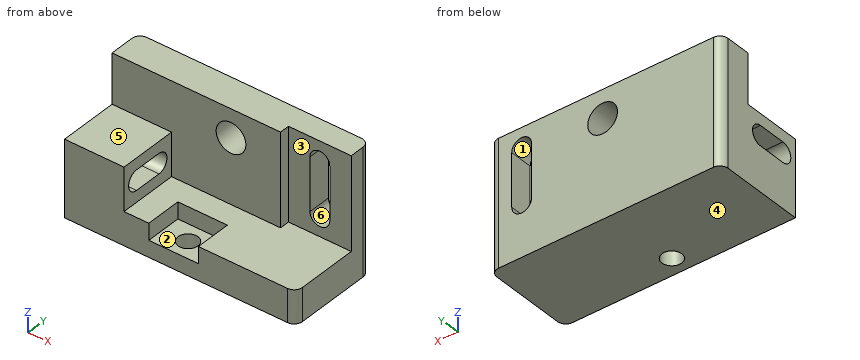
```python
from build123d import *

# Parameters (mm, degrees)
BASE_PLATE_DEPTH             = 76
SIDE_WALL_DEPTH              = 140
POCKET_PROFILE_W             = 38
POCKET_PROFILE_H             = 6
POCKET_CUT_DEPTH             = 56
SLOT_12X32_DEPTH             = 56
GUIDE_START                  = -36
GUIDE_RIB_DEPTH              = 36
OUTER_START                  = -140
OUTER_CORNER_ROUND_R10_DEPTH = 140
RIB_CORNER_ROUND_R10_DEPTH   = 104
CORNER_RELIEF_R10_DEPTH      = 104
HOLE_18_SKETCH_R             = 9
HOLE_18_DEPTH                = 104
NOTCH_PROFILE_W              = 30
NOTCH_PROFILE_H              = 22
NOTCH_CUT_DEPTH              = 10
HOLE_12_SKETCH_R             = 6
HOLE_12_DEPTH                = 10
RIB_SLOT_12_WIDE_DEPTH       = 36


with BuildPart() as part:
    # Base Plate Profile → Base Plate (new body)
    with BuildSketch(Plane.XY):
        with BuildLine():
            Line((5, 0), (135, 0))
            ThreePointArc((135, 0), (138.535533906, -1.464466094), (140, -5))
            Line((140, -5), (140, -20))
            Line((140, -20), (0, -20))
            Line((0, -20), (0, -5))
            ThreePointArc((0, -5), (1.464466094, -1.464466094), (5, 0))
        make_face()
    extrude(amount=BASE_PLATE_DEPTH)

    # Side Wall Profile → Side Wall (add)
    with BuildSketch(Plane(origin=(140, 0, 0), x_dir=(0, 0, -1), z_dir=(1, 0, 0))):
        with BuildLine():
            Line((0, -20), (0, -51))
            ThreePointArc((0, -51), (-1.464466094, -54.535533906), (-5, -56))
            Line((-5, -56), (-15, -56))
            ThreePointArc((-15, -56), (-18.535533906, -54.535533906), (-20, -51))
            Line((-20, -51), (-20, -20))
            Line((-20, -20), (0, -20))
        make_face()
    extrude(amount=-SIDE_WALL_DEPTH)

    # Pocket Profile → Pocket Cut (cut)
    with BuildSketch(Plane.XY.offset(76)):
        with Locations((121, -17)):
            Rectangle(POCKET_PROFILE_W, POCKET_PROFILE_H)
    extrude(amount=-POCKET_CUT_DEPTH, mode=Mode.SUBTRACT)

    # Slot 12x32 Profile → Slot 12x32 (cut)
    with BuildSketch(Plane.XZ.offset(14)):
        with BuildLine():
            Line((115, 64), (115, 32))
            ThreePointArc((115, 32), (121, 26), (127, 32))
            Line((127, 32), (127, 64))
            ThreePointArc((127, 64), (121, 70), (115, 64))
        make_face()
    extrude(amount=-SLOT_12X32_DEPTH, mode=Mode.SUBTRACT)

    # Guide Rib Profile → Guide Rib (add)
    with BuildSketch(Plane.ZY.offset(GUIDE_START)):
        with BuildLine():
            Line((20, -20), (46, -20))
            Line((46, -20), (46, -56))
            Line((46, -56), (15, -56))
            ThreePointArc((15, -56), (18.535533906, -54.535533906), (20, -51))
            Line((20, -51), (20, -20))
        make_face()
    extrude(amount=GUIDE_RIB_DEPTH)

    # Outer Corner Round Profile → Outer Corner Round R10 (add)
    with BuildSketch(Plane.ZY.offset(OUTER_START)):
        with BuildLine():
            Line((0, -51), (0, -56))
            Line((0, -56), (5, -56))
            ThreePointArc((5, -56), (1.464466094, -54.535533906), (0, -51))
        make_face()
    extrude(amount=OUTER_CORNER_ROUND_R10_DEPTH)

    # Rib Corner Round Profile → Rib Corner Round R10 (add)
    with BuildSketch(Plane(origin=(140, 0, 0), x_dir=(0, 0, -1), z_dir=(1, 0, 0))):
        with BuildLine():
            Line((-20, -51), (-20, -56))
            Line((-20, -56), (-15, -56))
            ThreePointArc((-15, -56), (-18.535533906, -54.535533906), (-20, -51))
        make_face()
    extrude(amount=-RIB_CORNER_ROUND_R10_DEPTH)

    # Corner Relief Profile → Corner Relief R10 (cut)
    with BuildSketch(Plane.XY.offset(20)):
        with BuildLine():
            Line((140, -56), (140, -51))
            ThreePointArc((140, -51), (138.535533906, -54.535533906), (135, -56))
            Line((135, -56), (140, -56))
        make_face()
    extrude(amount=-CORNER_RELIEF_R10_DEPTH, mode=Mode.SUBTRACT)

    # Hole Ø18 Sketch → Hole Ø18 (cut)
    with BuildSketch(Plane.XZ.offset(20)):
        with Locations(Location((72, 59, 0), (0, 0, 270))):
            Circle(HOLE_18_SKETCH_R)
    extrude(amount=-HOLE_18_DEPTH, mode=Mode.SUBTRACT)

    # Notch Profile → Notch Cut (cut)
    with BuildSketch(Plane.XY.offset(20)):
        with Locations((66, -45)):
            Rectangle(NOTCH_PROFILE_W, NOTCH_PROFILE_H)
    extrude(amount=-NOTCH_CUT_DEPTH, mode=Mode.SUBTRACT)

    # Hole Ø12 Sketch → Hole Ø12 (cut)
    with BuildSketch(Plane.XY.offset(10)):
        with Locations((66, -45)):
            Circle(HOLE_12_SKETCH_R)
    extrude(amount=-HOLE_12_DEPTH, mode=Mode.SUBTRACT)

    # Rib Slot Profile → Rib Slot 12 Wide (cut)
    with BuildSketch(Plane(origin=(36, 0, 0), x_dir=(0, 0, -1), z_dir=(1, 0, 0))):
        with BuildLine():
            Line((-39, -29.5), (-39, -46.5))
            ThreePointArc((-39, -46.5), (-33, -52.5), (-27, -46.5))
            Line((-27, -46.5), (-27, -29.5))
            ThreePointArc((-27, -29.5), (-33, -23.5), (-39, -29.5))
        make_face()
    extrude(amount=-RIB_SLOT_12_WIDE_DEPTH, mode=Mode.SUBTRACT)


solid = part.part
```
Can you work these out from the model? Positions are in its coordinate system, mm. Face numbers are marked on the shaded views. A direction names the side the tool comes from. Give positions to 0.01 mm unless a question says otherwise; leave off trailing zeros. Write each loop counter-clockwise with the first axis right and the second up, starting at its lowest first coordinate (ties: lowest second). Pieces come first, ordered by that corner, then holes. Notation, with made-up numbers: (-39.5, 25.5) - (-19.5, 25.5) arc R33 ccw to (-19.5, 58.5) - close; hole circle Ø3 at (6, 9). An arc over 180 degrees is marked (long way). Write item = value, one per line. Start each with the question number.
1. Imagine slicing it at A-A (z = 44.5). Please give me the cut outline in (x, y).
2. Imagine slicing it at D-D (y = -45). Please give me the cut outline in (x, z).
3. For pin 1 (17 mm diameter, centred on x = 72, z = 46.5, fed in from -Y); pin 2 (12 mm diameter, centred on y = -49, z = 31, fed in from +X); pin 3 (8 mm diameter, centred on x = 66.5, z = 15.5, fed in from -Y), each with a flat end and sliding along its axis, tell me the tip position at first contact or that it passes through.
4. On a 3-axis mill with a long thin cutter (end or side, diameter ignored), from which of +Z, -Z, +X, -X, +Y, -Y can I reach the whole of each face in a straight line? I mean the marked faces 1, 2 and 3. Say none if no direction works.
5. Please list where these lines run through material, in increasing order: line 1 (X direction, y = -7, z = 59); line 2 (X direction, y = -14.5, z = 59); line 3 (Y direction, x = 104, z = 54).
6. Thinking about a two-plate mould opening in Z: for the marked faces 4, 5 and 6, which applies, released by +Z, released by -Z, zero draft, split by the parting line, or undercut?
7. Imagine slicing it at C-C (x = 18.5). Please give me the cut outline in (y, z).
8. Imagine slicing it at B-B (y = -37). Please give me the cut outline in (x, z).
Worked answers:
q1.outline = (0, -56) - (36, -56) - (36, -20) - (102, -20) - (102, -14) - (115, -14) - (115, 0) - (5, 0) arc R5 ccw to (0, -5) - close; (127, -14) - (140, -14) - (140, -5) arc R5 ccw to (135, 0) - (127, 0) - close
q2.outline = (0, 0) - (60, 0) - (60, 10) - (51, 10) - (51, 20) - (36, 20) - (36, 27) - (0, 27) - close; (0, 39) - (36, 39) - (36, 46) - (0, 46) - close; (72, 0) - (140, 0) - (140, 20) - (81, 20) - (81, 10) - (72, 10) - close
q3.pin_1 = -20
q3.pin_2 = 36
q3.pin_3 = -34
q4.face_1 = +Y, -Y
q4.face_2 = +Z, -Y
q4.face_3 = +Z, +X, -Y
q5.line_1 = 0 to 63, 81 to 115, 127 to 140
q5.line_2 = 0 to 63, 81 to 102
q5.line_3 = -14 to 0
q6.face_4 = released by -Z
q6.face_5 = released by +Z
q6.face_6 = undercut
q7.outline = (-56, 0) - (0, 0) - (0, 76) - (-20, 76) - (-20, 46) - (-56, 46) - close; hole (-46.5, 27) - (-29.5, 27) arc R6 ccw to (-29.5, 39) - (-46.5, 39) arc R6 ccw to start
q8.outline = (0, 0) - (140, 0) - (140, 20) - (81, 20) - (81, 10) - (51, 10) - (51, 20) - (36, 20) - (36, 27) - (0, 27) - close; (0, 39) - (36, 39) - (36, 46) - (0, 46) - close
